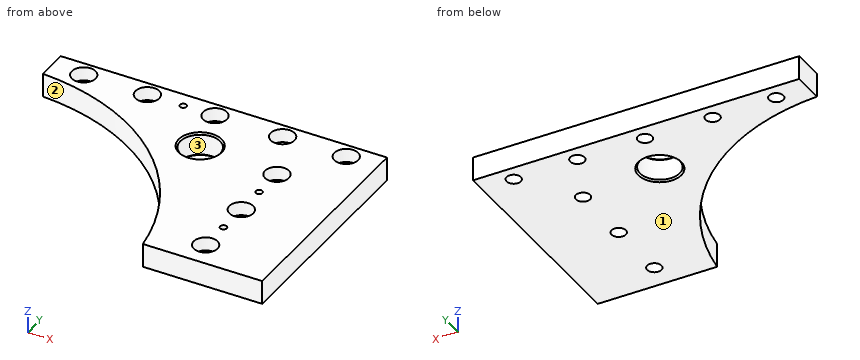
```python
from build123d import *

# Parameters (mm, degrees)
EXTRUDE_1_DEPTH              = 7.5
HOLE_WIZARD_M8_2_D           = 9
HOLE_WIZARD_M8_2_CBORE_D     = 15
HOLE_WIZARD_M8_2_CBORE_DEPTH = 8.6
HOLE_WIZARD_M5_1_D           = 4.2
HOLE_WIZARD_M5_1_DEPTH       = 12.4
HOLE_WIZARD_M5_1_TIP         = 1.2618073
SKETCH_11_R                  = 140
CUT_EXTRUDE_2_DEPTH          = 249.696602309
SKETCH_12_R                  = 12.5
CUT_EXTRUDE_3_DEPTH          = 326.153809758
CHAMFER_1_SIZE               = 1


with BuildPart() as part:
    # 草图1 → 凸台-拉伸1 (new, symmetric)
    with BuildSketch(Plane.XY):
        Polygon((0, 0), (205, 0), (205, -140), (130, -140), (0, -20), align=None)
    extrude(amount=EXTRUDE_1_DEPTH, both=True)

    # M8 六角凹头螺钉的柱形沉头孔2 (through all)
    with Locations(Plane.XY.offset(7.5)):
        with Locations((20, -10), (60, -10), (145, -10), (102.5, -10), (185, -10), (160.5, -44), (160.5, -84), (160.5, -124)):
            CounterBoreHole(HOLE_WIZARD_M8_2_D / 2, HOLE_WIZARD_M8_2_CBORE_D / 2, HOLE_WIZARD_M8_2_CBORE_DEPTH)

    # M5 螺纹孔1
    with Locations(Plane.XY.offset(7.5)):
        with Locations((82.5, -10), (143.75, -10), (160.5, -64), (160.5, -104)):
            Hole(HOLE_WIZARD_M5_1_D / 2, depth=HOLE_WIZARD_M5_1_DEPTH)
            with Locations((0, 0, -(HOLE_WIZARD_M5_1_DEPTH + HOLE_WIZARD_M5_1_TIP / 2))):  # 118° drill point
                Cone(0, HOLE_WIZARD_M5_1_D / 2, HOLE_WIZARD_M5_1_TIP, mode=Mode.SUBTRACT)

    # 草图11 → 切除-拉伸2 (cut, through all)
    with BuildSketch(Plane.XY.offset(7.5)):
        with Locations((-8.60198636, -159.735485224)):
            Circle(SKETCH_11_R)
    extrude(amount=-CUT_EXTRUDE_2_DEPTH, mode=Mode.SUBTRACT)

    # 草图12 → 切除-拉伸3 (cut, through all)
    with BuildSketch(Plane(origin=(0, 0, -202.5), x_dir=(-1, 0, 0), z_dir=(0, 0, -1))):
        with Locations((-110, -40)):
            Circle(SKETCH_12_R)
    extrude(amount=-CUT_EXTRUDE_3_DEPTH, mode=Mode.SUBTRACT)

    # 倒角1
    chamfer_1_edges = [part.edges().sort_by_distance(p)[0] for p in [
        (122.5, -40, 7.5),
        (122.5, -40, -7.5),
    ]]
    chamfer(chamfer_1_edges, length=CHAMFER_1_SIZE)


solid = part.part
```
Can you work these out from the model? Positions are in its coordinate system, mm. Face numbers are marked on the shaded views. Coordinates: 2 decimals unless noted, no trailing zeros. Write each loop counter-clockwise with the first axis right and the second up, starting at its lowest first coordinate (ties: lowest second). Pieces come first, ordered by that corner, then holes. Notation, with made-up numbers: (84.25, 33) - (135.25, 33) arc R22 ccw to (135.25, 47) - close; hole circle Ø7 at (37.25, -28.5). An arc over 180 degrees is marked (long way). Return JSON: item names as keys, results as strings.
Q1. Please list where these lines run through material, in increasing order: L1, parallel to Y at x = 160.5, z = 0; L2, parallel to Y at x = 102.5, z = -4.75; L3, parallel to Y at x = 98.5, z = -5. Write a range as from..to.
Computed values:
{"L1": "y = -140..-131.5, -116.5..-106.1, -101.9..-91.5, -76.5..-66.1, -61.9..-51.5, -36.5..0", "L2": "y = -74.55..-50, -30..-14.5, -5.5..0", "L3": "y = -69.57..-44.9, -35.1..-12.06, -7.94..0"}
Q2. If we section it at C-C (x = 60): Please give me the cut outline in (y, z).
Computed values:
{"outline": "(-37.7, -7.5) - (-14.5, -7.5) - (-14.5, -1.1) - (-17.5, -1.1) - (-17.5, 7.5) - (-37.7, 7.5) - close; (-5.5, -7.5) - (0, -7.5) - (0, 7.5) - (-2.5, 7.5) - (-2.5, -1.1) - (-5.5, -1.1) - close"}
Q3. If we section it at D-D (x = 91.5): Please give me the cut outline in (y, z).
Computed values:
{"outline": "(-61.86, -7.5) - (0, -7.5) - (0, 7.5) - (-61.86, 7.5) - close"}
Q4. Thinking about a two-plate mould opening in Y: for the marked faces 1, 2 and 3, which applies, +Y half, -Y half, draft (parallel to the pull), parting line (faces both ways), or undercut?
Computed values:
{"face 1": "draft", "face 2": "-Y half", "face 3": "undercut"}
Q5. I'm going to push flat-ended pins straight in: pin 1 Ø12 at (x, y) = (20, -10) entering from +Z; pin 2 Ø6 at (y, z) = (-37, 1.5) entering from -X; pin 3 Ø5.5 at (x, y) = (60, -10) entering from +Z; pin 4 Ø1 at (y, z) = (-96, -3) entering from -X. Where does each tip first touch, or does it pass through?
Computed values:
{"pin 1": "stops at z = -1.1", "pin 2": "stops at x = 52.97", "pin 3": "passes through", "pin 4": "stops at x = 115.79"}
Q6. If we section it at B-B (y = -84): Please give me the cut outline in (x, z).
Computed values:
{"outline": "(109.14, -7.5) - (156, -7.5) - (156, -1.1) - (153, -1.1) - (153, 7.5) - (109.14, 7.5) - close; (165, -7.5) - (205, -7.5) - (205, 7.5) - (168, 7.5) - (168, -1.1) - (165, -1.1) - close"}
Q7. If we section it at A-A (z = 3): Count the separate pieces of the cut face and the enclosed holes in it, then the cut area to 3 significant figures.
Computed values:
{"separate pieces": "1", "enclosed holes": "12", "area": "15,100 mm2"}
